from build123d import *

# Parameters (mm, degrees)
SKETCH1_W             = 50
SKETCH1_H             = 20
BOSS_EXTRUDE1_DEPTH   = 100
SKETCH2_R             = 3
BOSS_EXTRUDE2_DEPTH   = 5
M6_TAPPED_HOLE1_D     = 5
M6_TAPPED_HOLE1_DEPTH = 15
M6_TAPPED_HOLE1_TIP   = 1.502151548
SKETCH5_W             = 20
SKETCH5_H             = 30
BOSS_EXTRUDE3_DEPTH   = 120
M3_TAPPED_HOLE1_D     = 2.5
M3_TAPPED_HOLE1_DEPTH = 7.5
M3_TAPPED_HOLE1_TIP   = 0.751075774
SKETCH8_W             = 95.008103892
SKETCH8_H             = 183.237528091
CUT_EXTRUDE1_DEPTH    = 163.249807396
CUT_EXTRUDE2_DEPTH    = 101.124921973
SKETCH10_W            = 120
SKETCH10_H            = 10
CUT_EXTRUDE3_DEPTH    = 163.249807396


with BuildPart() as part:
    # Sketch1 → Boss-Extrude1 (new body)
    with BuildSketch(Plane(origin=(0, 0, 0), x_dir=(1, 0, 0), z_dir=(0, 1, 0))):
        Rectangle(SKETCH1_W, SKETCH1_H)
    extrude(amount=BOSS_EXTRUDE1_DEPTH)

    # Sketch2 → Boss-Extrude2 (add)
    with BuildSketch(Plane.XZ):
        with Locations(Location((0, 5, 0), (0, 0, 270))):
            Circle(SKETCH2_R)
    extrude(amount=BOSS_EXTRUDE2_DEPTH)

    # M6 Tapped Hole1
    with Locations(Plane(origin=(0, 0, 0), x_dir=(-1, 0, 0), z_dir=(0, -1, 0))):
        with Locations((0, 5)):
            Hole(M6_TAPPED_HOLE1_D / 2, depth=M6_TAPPED_HOLE1_DEPTH)
            with Locations((0, 0, -(M6_TAPPED_HOLE1_DEPTH + M6_TAPPED_HOLE1_TIP / 2))):  # 118° drill point
                Cone(0, M6_TAPPED_HOLE1_D / 2, M6_TAPPED_HOLE1_TIP, mode=Mode.SUBTRACT)

    # Sketch5 → Boss-Extrude3 (add)
    with BuildSketch(Plane(origin=(25, 0, 0), x_dir=(0, 0, -1), z_dir=(1, 0, 0))):
        with Locations((0, 115)):
            Rectangle(SKETCH5_W, SKETCH5_H)
    extrude(amount=-BOSS_EXTRUDE3_DEPTH)

    # M3 Tapped Hole1
    with Locations(Plane.XY.offset(10)):
        with Locations((-63.4, 108), (-59.4, 112), (-67.4, 105)):
            Hole(M3_TAPPED_HOLE1_D / 2, depth=M3_TAPPED_HOLE1_DEPTH)
            with Locations((0, 0, -(M3_TAPPED_HOLE1_DEPTH + M3_TAPPED_HOLE1_TIP / 2))):  # 118° drill point
                Cone(0, M3_TAPPED_HOLE1_D / 2, M3_TAPPED_HOLE1_TIP, mode=Mode.SUBTRACT)

    # Sketch8 → Cut-Extrude1 (cut, through all)
    with BuildSketch(Plane.XY.offset(10)):
        with Locations((22.504051946, 8.381235954)):
            Rectangle(SKETCH8_W, SKETCH8_H)
    extrude(amount=-CUT_EXTRUDE1_DEPTH, mode=Mode.SUBTRACT)

    # Sketch9 → Cut-Extrude2 (cut, through all)
    with BuildSketch(Plane(origin=(0, 130, 0), x_dir=(1, 0, 0), z_dir=(0, 1, 0))):
        with BuildLine():
            Line((10.388294344, -3.2), (-19.611705656, -3.2))
            ThreePointArc((-19.611705656, -3.2), (-22.811705656, 0), (-19.611705656, 3.2))
            Line((-19.611705656, 3.2), (10.388294344, 3.2))
            ThreePointArc((10.388294344, 3.2), (13.588294344, 0), (10.388294344, -3.2))
        make_face()
    extrude(amount=-CUT_EXTRUDE2_DEPTH, mode=Mode.SUBTRACT)

    # Sketch10 → Cut-Extrude3 (cut, through all)
    with BuildSketch(Plane.XY.offset(10)):
        with Locations((-35, 125)):
            Rectangle(SKETCH10_W, SKETCH10_H)
    extrude(amount=-CUT_EXTRUDE3_DEPTH, mode=Mode.SUBTRACT)


solid = part.part
Geometry check sheet. Reference: the model listing, model coordinates, mm. A direction names the side the tool comes from. Coordinates: 2 decimals unless noted, no trailing zeros. Order: outer loops, then holes, each group sorted by start corner. A loop starts at its lowest first (then second) coordinate and runs counter-clockwise, first axis right, second up. Notation, with made-up numbers: (16, 37.5) - (26, 37.5) arc R18 cw to (26, 49.5) - close; hole circle Ø5 at (10, 77). An arc over 180 degrees is marked (long way). One line per item, written item: value.
(1) Sectioned sample at A-A (z = 0). Enter the section's corners in (x, y), and give its area (3 significant figures).
Data:
outline: (-95, 100) - (-22.81, 100) - (-22.81, 120) - (-95, 120) - close; (13.59, 100) - (25, 100) - (25, 120) - (13.59, 120) - close
area: 1,670 mm^2
(2) Access from +Z, -Z, +X, -X, +Y, -Y to the whole of each face (thin tool, end or side, straight path). Record for faces 5 (the face through (-63.24, 109.24, 6.2)), 6 (the face through (25, 110, 0)), 7 (the face through (13.588, 110.14, -0.07)).
Data:
face 5: +Z
face 6: +Z, -Z, +X, +Y, -Y
face 7: +Y, -Y
(3) Release check for a two-part mould opening along Y. For faces 1 (the face through (-95, 110, 0)), 2 (the face through (-67.24, 106.24, 6.2)), 3 (the face through (-63.428, 108.215, 1.879)), 4 (the face through (-36, 100, 0)) record: +Y half, -Y half, draft (parallel to the pull), parting line (faces both ways), or undercut.
Data:
face 1: draft
face 2: undercut
face 3: undercut
face 4: -Y half
(4) Thickness scan on probe 1 along Z at (x, y) = (-2, 115.5); probe 2 along X at (y, z) = (105, 5); probe 3 along Y at (x, z) = (-59.4, 7.5). Record the ranges inside material, lowest first. Write a range as from..to.
Data:
probe 1: z = -10..-3.2, 3.2..10
probe 2: x = -95..-68.65, -66.15..25
probe 3: y = 100..110.75, 113.25..120
(5) Depth check by flat-ended pin: pin 1 Ø2 at (x, y) = (-67.4, 105) entering from +Z. Enter the tip coordinate at first touch or a pass-through.
Data:
pin 1: stops at z = 2.35
(6) Sectioned sample at B-B (x = -16). Enter the section's corners in (y, z).
Data:
outline: (100, -10) - (120, -10) - (120, -3.2) - (100, -3.2) - close; (100, 3.2) - (120, 3.2) - (120, 10) - (100, 10) - close
